from build123d import *

# Parameters (mm, degrees)
SKETCH1_R           = 2.5
BOSS_EXTRUDE1_DEPTH = 50
CUT_EXTRUDE1_DEPTH  = 5
CUT_EXTRUDE3_START  = -12
CUT_EXTRUDE3_DEPTH  = 12


with BuildPart() as part:
    # Sketch1 → Boss-Extrude1 (new body)
    with BuildSketch(Plane.XY):
        Circle(SKETCH1_R)
    extrude(amount=BOSS_EXTRUDE1_DEPTH)

    # Sketch2 → Cut-Extrude1 (cut)
    with BuildSketch(Plane(origin=(0, 0, 0), x_dir=(-1, 0, 0), z_dir=(0, 0, -1))):
        with BuildLine():
            Line((-1.835, 1.69787367), (1.835, 1.69787367))
            ThreePointArc((1.835, 1.69787367), (0, 2.5), (-1.835, 1.69787367))
        make_face()
    extrude(amount=-CUT_EXTRUDE1_DEPTH, mode=Mode.SUBTRACT)

    # Sketch3 → Cut-Extrude3 (cut)
    with BuildSketch(Plane.XY.offset(50).offset(CUT_EXTRUDE3_START)):
        with BuildLine():
            Line((-1.835, 1.69787367), (1.835, 1.69787367))
            ThreePointArc((1.835, 1.69787367), (0, 2.5), (-1.835, 1.69787367))
        make_face()
    extrude(amount=CUT_EXTRUDE3_DEPTH, mode=Mode.SUBTRACT)


solid = part.part
The model under review builds one solid part; all positions refer to its coordinate system, in mm. A direction names the side the tool comes from. Round coordinates to 2 decimals unless told otherwise and drop trailing zeros. Loops run counter-clockwise (first coordinate to the right, second up) from the corner with the lowest first, then second, coordinate; pieces in that order, holes last. Notation, with made-up numbers: M 27.5,82.25 L 36.5,82.25 A22 ccw 36.5,103.25 Z; hole C 33.25,1.5 d8. An arc over 180 degrees is marked long. Answer as CSV lines item,"result".
1. We need section D-D (z = 5.5). Give the boundary of the cut face in (x, y), plus the area to 3 significant figures.
Outcome:
outline,"C 0,0 d5"
area,"19.6 mm2"
2. We need section C-C (y = -1). Give the boundary of the cut face in (x, z).
Outcome:
outline,"M -2.29,0 L 2.29,0 L 2.29,50 L -2.29,50 Z"
3. We need section B-B (z = 43.5). Give the boundary of the cut face in (x, y) (3 decimals).
Outcome:
outline,"M -1.835,1.698 A2.5 ccw long 1.835,1.698 Z"
4. To check wall thickness, follow L1, parallel to X at y = 1.35, z = 44; L2, parallel to X at y = -0.35, z = 28; L3, parallel to Y at x = 0.6, z = 42.5. State the ranges of each line that lie inside material, in increasing order. Write a range as [from, to].
Outcome:
L1,"x = [-2.1, 2.1]"
L2,"x = [-2.48, 2.48]"
L3,"y = [-2.43, 1.7]"
5. We need section A-A (x = 0). Give the boundary of the cut face in (y, z), plus the area to 3 significant figures.
Outcome:
outline,"M -2.5,0 L 1.7,0 L 1.7,5 L 2.5,5 L 2.5,38 L 1.7,38 L 1.7,50 L -2.5,50 Z"
area,"236 mm2"
6. For faces 1 (the face through (0, 2, 38)), 2 (the face through (-0.54, -2.44, 24.65)), 3 (the face through (0, 2, 5)), list the 3-axis set-ups (+Z, -Z, +X, -X, +Y, -Y) from which the entire face can be reached by the end or side of a thin tool; tool diameter is ignored.
Outcome:
face 1,"+Z, +X, -X, +Y"
face 2,"+Z, -Z"
face 3,"-Z, +X, -X, +Y"
7. Insertion check: pin 1 Ø1.5 at (y, z) = (-1.5, 40) entering from -X; pin 2 Ø1 at (x, z) = (-1.5, 7) entering from -Y; pin 3 Ø1.1 at (x, z) = (-0.5, 44) entering from +Y. Each pin has a flat end and moves straight along its axis. Give the tip position at first contact, or say it passes through.
Outcome:
pin 1,"stops at x = -2.38"
pin 2,"stops at y = -2.29"
pin 3,"stops at y = 1.7"
